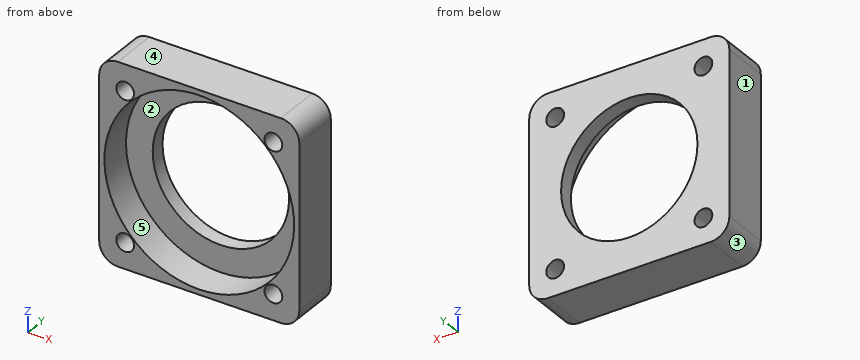
```python
from build123d import *

# Parameters (mm, degrees)
BASE_PLATE_PROFILE_R        = 6
BASE_PLATE_135X135X32_DEPTH = 32
THROUGH_BORE_92_REACH       = 102.68
THROUGH_BORE_PROFILE_R      = 46
COUNTERBORE_PROFILE_R       = 64
COUNTERBORE_128X22_DEPTH    = 22


with BuildPart() as part:
    # Base Plate Profile → Base Plate 135x135x32 (new body)
    with BuildSketch(Plane(origin=(0, 0, 0), x_dir=(1, 0, 0), z_dir=(0, 1, 0))):
        with BuildLine():
            Line((-55, 67.5), (55, 67.5))
            ThreePointArc((55, 67.5), (63.838834765, 63.838834765), (67.5, 55))
            Line((67.5, 55), (67.5, -55))
            ThreePointArc((67.5, -55), (63.838834765, -63.838834765), (55, -67.5))
            Line((55, -67.5), (-55, -67.5))
            ThreePointArc((-55, -67.5), (-63.838834765, -63.838834765), (-67.5, -55))
            Line((-67.5, -55), (-67.5, 55))
            ThreePointArc((-67.5, 55), (-63.838834765, 63.838834765), (-55, 67.5))
        make_face()
        with Locations(Location((-50, 50, 0), (0, 0, 270))):
            Circle(BASE_PLATE_PROFILE_R, mode=Mode.SUBTRACT)
        with Locations(Location((50, 50, 0), (0, 0, 90))):
            Circle(BASE_PLATE_PROFILE_R, mode=Mode.SUBTRACT)
        with Locations(Location((50, -50, 0), (0, 0, 270))):
            Circle(BASE_PLATE_PROFILE_R, mode=Mode.SUBTRACT)
        with Locations(Location((-50, -50, 0), (0, 0, 90))):
            Circle(BASE_PLATE_PROFILE_R, mode=Mode.SUBTRACT)
    extrude(amount=BASE_PLATE_135X135X32_DEPTH)

    # Through Bore Profile → Through Bore Ø92 (cut, up to next)
    with BuildSketch(Plane(origin=(0, 32, 0), x_dir=(1, 0, 0), z_dir=(0, 1, 0)), mode=Mode.PRIVATE) as through_bore_92_sk1:
        with Locations(Location((0, 0, 0), (0, 0, 270))):
            Circle(THROUGH_BORE_PROFILE_R)
    through_bore_92_tool1 = extrude(through_bore_92_sk1.sketch, amount=-THROUGH_BORE_92_REACH, mode=Mode.PRIVATE) & part.part
    add(through_bore_92_tool1.solids().sort_by_distance((0, 32, 0))[0], mode=Mode.SUBTRACT)

    # Counterbore Profile → Counterbore Ø128x22 (cut)
    with BuildSketch(Plane(origin=(0, 0, 0), x_dir=(-1, 0, 0), z_dir=(0, -1, 0))):
        with Locations(Location((0, 0, 0), (0, 0, 90))):
            Circle(COUNTERBORE_PROFILE_R)
    extrude(amount=-COUNTERBORE_128X22_DEPTH, mode=Mode.SUBTRACT)


solid = part.part
```
Geometry: final body of the model. Coordinates: model frame, mm. Face numbers are marked on the shaded views. A direction names the side the tool comes from. Round coordinates to 2 decimals unless told otherwise and drop trailing zeros. Write each loop counter-clockwise with the first axis right and the second up, starting at its lowest first coordinate (ties: lowest second). Pieces come first, ordered by that corner, then holes.
Item 1: Material intervals for L1, parallel to X at y = 24, z = -50; L2, parallel to X at y = 17.5, z = 1.5; L3, parallel to X at y = 25, z = -54, sorted ascending.
Item 2: Set-up query: the marked faces 4 and 5. Return all of +Z, -Z, +X, -X, +Y, -Y with unobstructed straight access to the full face (end or side cutting, diameter ignored); none if empty.
Item 3: Section query B-B (z = 0). Return loops of the section in (x, y), plus the area to 3 significant figures.
Item 4: Section query D-D (z = -50). Return loops of the section in (x, y), plus the area to 3 significant figures.
Item 5: Section query C-C (y = 10). Return loops of the section in (x, z), plus the area to 3 significant figures.
Item 6: Section query A-A (x = 0). Return loops of the section in (y, z), plus the area to 3 significant figures.
Item 7: Pin query (flat end, axial travel): P1, Ø7, axis at x = 50, z = -50, coming from the -Y side; P2, Ø5, axis at x = -29, z = -49, coming from the -Y side. Return the tip coordinate at first contact, or that it passes through.
Item 8: Mould query, pull axis Z, two halves, no side actions, for the marked faces 1, 2 and 3. Classes: +Z half, -Z half, draft (parallel to the pull), parting line (faces both ways), or undercut.
Completed:
1. L1: x = -67.5 to -56, -44 to 44, 56 to 67.5
1. L2: x = -67.5 to -63.98, 63.98 to 67.5
1. L3: x = -67.5 to -54.47, -45.53 to 45.53, 54.47 to 67.5
2. face 4: +Z, +X, -X, +Y, -Y
2. face 5: -Y
3. outline: (-67.5, 0) - (-64, 0) - (-64, 22) - (-46, 22) - (-46, 32) - (-67.5, 32) - close; (46, 22) - (64, 22) - (64, 0) - (67.5, 0) - (67.5, 32) - (46, 32) - close
3. area: 584 mm2
4. outline: (-67.5, 0) - (-56, 0) - (-56, 32) - (-67.5, 32) - close; (-44, 0) - (-39.95, 0) - (-39.95, 22) - (39.95, 22) - (39.95, 0) - (44, 0) - (44, 32) - (-44, 32) - close; (56, 0) - (67.5, 0) - (67.5, 32) - (56, 32) - close
4. area: 1,790 mm2
5. outline: (-67.5, -55) arc R12.5 ccw to (-55, -67.5) - (55, -67.5) arc R12.5 ccw to (67.5, -55) - (67.5, 55) arc R12.5 ccw to (55, 67.5) - (-55, 67.5) arc R12.5 ccw to (-67.5, 55) - close; hole circle Ø128 at (0, 0); hole circle Ø12 at (-50, -50); hole circle Ø12 at (-50, 50); hole circle Ø12 at (50, -50); hole circle Ø12 at (50, 50)
5. area: 4,770 mm2
6. outline: (0, -67.5) - (32, -67.5) - (32, -46) - (22, -46) - (22, -64) - (0, -64) - close; (0, 64) - (22, 64) - (22, 46) - (32, 46) - (32, 67.5) - (0, 67.5) - close
6. area: 584 mm2
7. P1: passes through
7. P2: stops at y = 22
8. face 1: draft
8. face 2: undercut
8. face 3: -Z half
